Could you check a few things on this drawing? It's one solid part, dimensions in mm from its lowest x, y, z. Give positions to 0.01 mm unless a question says otherwise; leave off trailing zeros. Write each loop counter-clockwise with the first axis right and the second up, starting at its lowest first coordinate (ties: lowest second). Pieces come first, ordered by that corner, then holes.
1. Suppose I cut it at C-C (y = 1.1). Please give me the cut outline in (x, z) (3 decimals), and give its area (3 significant figures).
2. Suppose I cut it at D-D (z = 23.5). Please give me the cut outline in (x, y), and give its area (3 significant figures).
3. I'm going to push flat-ended pins straight in: pin 1 (1.5 mm diameter, centred on y = 3, z = 21, fed in from +X); pin 2 (5 mm diameter, centred on x = 91.63, z = 91.63, fed in from +Y). Where does each tip first touch, or does it pass through?
4. Suppose I cut it at B-B (z = 10). Please give me the cut outline in (x, y), and give its area (3 significant figures).
5. If I drill on probe 1 along X at (y, z) = (1.8, 94); probe 2 along Z at (x, y) = (10, 1.85), over which ranges is the centre line in solid material (lowest first)?
6. Suppose I cut it at A-A (x = 7.5). Please give me the cut outline in (y, z).
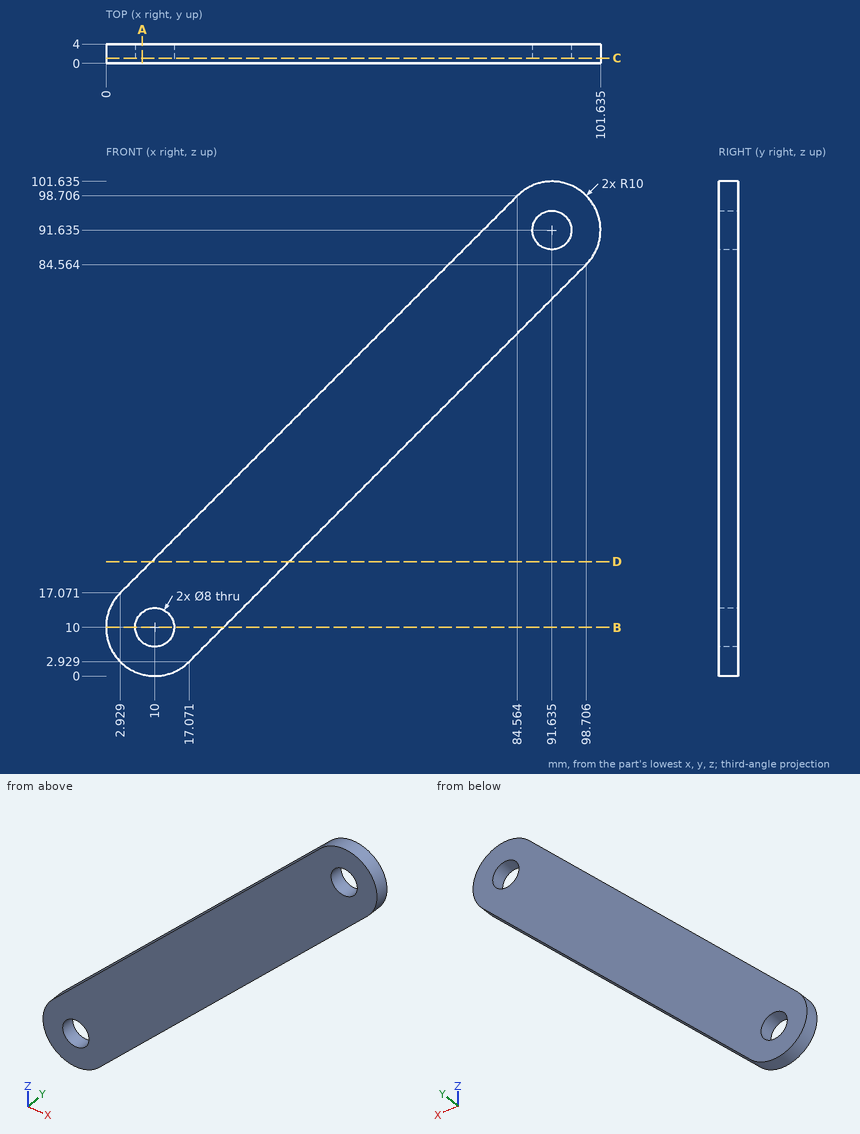
Checks:
1. outline: (2.929, 17.071) arc R10 ccw to (17.071, 2.929) - (98.706, 84.564) arc R10 ccw to (84.564, 98.706) - close; hole circle Ø8 at (10, 10); hole circle Ø8 at (91.635, 91.635)
1. area: 2,520 mm2
2. outline: (9.36, 0) - (37.64, 0) - (37.64, 4) - (9.36, 4) - close
2. area: 113 mm2
3. pin 1: stops at x = 35.89
3. pin 2: passes through
4. outline: (0, 0) - (6, 0) - (6, 4) - (0, 4) - close; (14, 0) - (24.14, 0) - (24.14, 4) - (14, 4) - close
4. area: 64.6 mm2
5. probe 1: x = 79.86 to 88.41, 94.86 to 101.35
5. probe 2: z = 0 to 6, 14 to 24.14
6. outline: (0, 0.32) - (4, 0.32) - (4, 6.88) - (0, 6.88) - close; (0, 13.12) - (4, 13.12) - (4, 21.64) - (0, 21.64) - close
